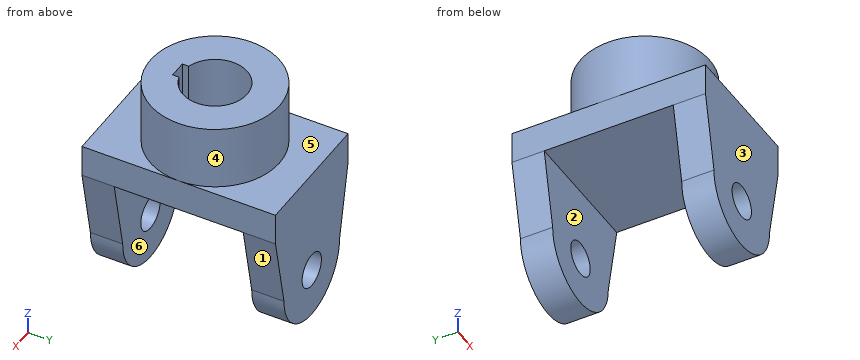
from build123d import *

# Parameters (mm, degrees)
SKETCH1_W           = 60
SKETCH1_H           = 90
BOSS_EXTRUDE1_DEPTH = 15
SKETCH2_R           = 8
BOSS_EXTRUDE2_DEPTH = 15
SKETCH3_R           = 30
BOSS_EXTRUDE3_DEPTH = 30


with BuildPart() as part:
    # Sketch1 → Boss-Extrude1 (new body)
    with BuildSketch(Plane.XY):
        Rectangle(SKETCH1_W, SKETCH1_H)
    extrude(amount=-BOSS_EXTRUDE1_DEPTH)

    # Sketch2 → Boss-Extrude2 (add)
    with BuildSketch(Plane(origin=(0, 45, 0), x_dir=(1, 0, 0), z_dir=(0, 1, 0))):
        with BuildLine():
            Line((-23, 50), (-30, 15))
            Line((-30, 15), (30, 15))
            Line((30, 15), (23, 50))
            ThreePointArc((23, 50), (0, 73), (-23, 50))
        make_face()
        with Locations(Location((0, 50, 0), (0, 0, 270))):
            Circle(SKETCH2_R, mode=Mode.SUBTRACT)
    boss_extrude2 = extrude(amount=-BOSS_EXTRUDE2_DEPTH)

    # Mirror1: Boss-Extrude2 across plane
    add(boss_extrude2.mirror(Plane.ZX))

    # Sketch3 → Boss-Extrude3 (add)
    with BuildSketch(Plane.XY):
        Circle(SKETCH3_R)
        with BuildLine():
            Line((-4, -14.456832295), (-4, -17.456832295))
            Line((-4, -17.456832295), (4, -17.456832295))
            Line((4, -17.456832295), (4, -14.456832295))
            ThreePointArc((4, -14.456832295), (0, 15), (-4, -14.456832295))
        make_face(mode=Mode.SUBTRACT)
    extrude(amount=BOSS_EXTRUDE3_DEPTH)


solid = part.part
Here's how the part is built. I have some questions about the finished solid (model axes, mm). Face numbers are marked on the shaded views. A direction names the side the tool comes from. Round coordinates to 2 decimals unless told otherwise and drop trailing zeros. Order: outer loops, then holes, each group sorted by start corner. A loop starts at its lowest first (then second) coordinate and runs counter-clockwise, first axis right, second up. Notation, with made-up numbers: (78.25, 3.25) -> (108.25, 3.25) arc R31 ccw to (108.25, 31.25) -> close; hole circle Ø3 at (1.5, 82.5). An arc over 180 degrees is marked (long way). Use CSV: the item, a comma, the result in double quotes.
1. I'm going to push flat-ended pins straight in: P1, Ø14.5, axis at x = 0, z = -50, coming from the -Y side; P2, Ø2, axis at x = -8.5, y = -13, coming from the -Z side; P3, Ø4, axis at x = 19, z = 7, coming from the -Y side; P4, Ø3, axis at x = 24, y = -23.5, coming from the +Z side. Where does each tip first touch, or does it pass through?
Recorded:
P1,"passes through"
P2,"stops at z = -15"
P3,"stops at y = -24.72"
P4,"stops at z = 0"
2. I want a section at A-A on z = -33. List the corners of the cut face in (x, y) for me, and give its area (3 significant figures).
Recorded:
outline,"(-26.4, -45) -> (26.4, -45) -> (26.4, -30) -> (-26.4, -30) -> close; (-26.4, 30) -> (26.4, 30) -> (26.4, 45) -> (-26.4, 45) -> close"
area,"1,580 mm2"
3. Which directions (+Z, -Z, +X, -X, +Y, -Y) give clear straight access to the entire face, cutting with the end or side of a thin tool? Please do the marked faces 4, 5 and 6.
Recorded:
face 4,"+Z"
face 5,"+Z, +Y"
face 6,"-Z, +X, -X"
4. I want a section at D-D on y = 23.5. List the corners of the cut face in (x, z) for me, and give its area (3 significant figures).
Recorded:
outline,"(-30, -15) -> (30, -15) -> (30, 0) -> (18.65, 0) -> (18.65, 30) -> (-18.65, 30) -> (-18.65, 0) -> (-30, 0) -> close"
area,"2,020 mm2"
5. I want a section at B-B on x = 0. List the corners of the cut face in (y, z) for me, and give its area (3 significant figures).
Recorded:
outline,"(-45, -73) -> (-30, -73) -> (-30, -58) -> (-45, -58) -> close; (-45, -42) -> (-30, -42) -> (-30, -15) -> (30, -15) -> (30, -42) -> (45, -42) -> (45, 0) -> (30, 0) -> (30, 30) -> (15, 30) -> (15, 0) -> (-17.46, 0) -> (-17.46, 30) -> (-30, 30) -> (-30, 0) -> (-45, 0) -> close; (30, -73) -> (45, -73) -> (45, -58) -> (30, -58) -> close"
area,"3,440 mm2"
6. I need wall thicknesses on line 1 along Y through (x, z) = (-14.5, -54.5); line 2 along X through (y, z) = (-36.75, -50); line 3 along Z through (x, y) = (0, -29). Which ranges of each line are inside material? Lowest first, please.
Recorded:
line 1,"y = -45 to -30, 30 to 45"
line 2,"x = -23 to -8, 8 to 23"
line 3,"z = -15 to 30"
7. Thinking about a two-plate mould opening in Y: for the marked faces 1, 2 and 3, which applies, pulls with the +Y half, pulls with the -Y half, needs draft (parallel to the pull), parting line crosses it, or undercut?
Recorded:
face 1,"needs draft"
face 2,"undercut"
face 3,"pulls with the -Y half"
8. I want a section at C-C on z = -48.5. List the corners of the cut face in (x, y) for me.
Recorded:
outline,"(-23.3, -45) -> (-7.86, -45) -> (-7.86, -30) -> (-23.3, -30) -> close; (-23.3, 30) -> (-7.86, 30) -> (-7.86, 45) -> (-23.3, 45) -> close; (7.86, -45) -> (23.3, -45) -> (23.3, -30) -> (7.86, -30) -> close; (7.86, 30) -> (23.3, 30) -> (23.3, 45) -> (7.86, 45) -> close"
